CAD build for the part. Positions are in the model's coordinates, mm. Face numbers are marked on the shaded views. A direction names the side the tool comes from. Coordinates: 2 decimals unless noted, no trailing zeros. Order: outer loops, then holes, each group sorted by start corner. A loop starts at its lowest first (then second) coordinate and runs counter-clockwise, first axis right, second up. Notation, with made-up numbers: M 73,88 L 99,88 A16 cw 99,111 Z; hole C 81,35 d6. An arc over 180 degrees is marked long. Write item = value, one per line. Start each with the question number.
```python
from build123d import *

# Parameters (mm, degrees)
HUB_SKETCH_20_R            = 10
HUB_CYLINDER_20_DEPTH      = 20
FIRST_START                = -20
FIRST_ARM_DEPTH            = 20
SECOND_START               = -20
SECOND_ARM_DEPTH           = 20
TAB_A_DEPTH                = 2.5
TAB_B_DEPTH                = 2.5
TAB_B_HOLE_SKETCH_10_R     = 5
TAB_B_HOLE_10_DEPTH        = 2.5
TAB_A_HOLE_SKETCH_10_R     = 5
TAB_A_HOLE_10_DEPTH        = 2.5
HUB_CROSS_BORE_SKETCH_10_R = 5
HUB_CROSS_BORE_10_DEPTH    = 20


with BuildPart() as part:
    # Hub Sketch Ø20 → Hub Cylinder Ø20 (new body)
    with BuildSketch(Plane.XY):
        Circle(HUB_SKETCH_20_R)
    extrude(amount=HUB_CYLINDER_20_DEPTH)

    # First Arm Sketch → First Arm (add)
    with BuildSketch(Plane.XY.offset(20).offset(FIRST_START)):
        with BuildLine():
            Line((0, 10), (25, 10))
            Line((25, 10), (25, 7.5))
            Line((25, 7.5), (6.614378278, 7.5))
            ThreePointArc((6.614378278, 7.5), (3.535533906, 9.354143467), (0, 10))
        make_face()
        with BuildLine():
            Line((0, -10), (-25, -10))
            Line((-25, -10), (-25, -7.5))
            Line((-25, -7.5), (-6.614378278, -7.5))
            ThreePointArc((-6.614378278, -7.5), (-3.535533906, -9.354143467), (0, -10))
        make_face()
    extrude(amount=FIRST_ARM_DEPTH)

    # Second Arm Sketch → Second Arm (add)
    with BuildSketch(Plane.XY.offset(20).offset(SECOND_START)):
        with BuildLine():
            ThreePointArc((-9.860132972, -1.666666667), (-10.971386379, -5.727486122), (-14.790199458, -7.5))
            Line((-14.790199458, -7.5), (-6.614378278, -7.5))
            ThreePointArc((-6.614378278, -7.5), (-8.738382269, -4.86216776), (-9.860132972, -1.666666667))
        make_face()
        with BuildLine():
            ThreePointArc((9.860132972, 1.666666667), (10.971386379, 5.727486122), (14.790199458, 7.5))
            Line((14.790199458, 7.5), (6.614378278, 7.5))
            ThreePointArc((6.614378278, 7.5), (8.738382269, 4.86216776), (9.860132972, 1.666666667))
        make_face()
    extrude(amount=SECOND_ARM_DEPTH)

    # Tab A Sketch → Tab A (add)
    with BuildSketch(Plane.XZ.offset(10)):
        with BuildLine():
            Line((-25, 20), (-25, 0))
            ThreePointArc((-25, 0), (-35, 10), (-25, 20))
        make_face()
    extrude(amount=-TAB_A_DEPTH)

    # Tab B Sketch → Tab B (add)
    with BuildSketch(Plane(origin=(0, 10, 0), x_dir=(1, 0, 0), z_dir=(0, 1, 0))):
        with BuildLine():
            Line((25, 0), (25, -20))
            ThreePointArc((25, -20), (35, -10), (25, 0))
        make_face()
    extrude(amount=-TAB_B_DEPTH)

    # Tab B Hole Sketch Ø10 → Tab B Hole Ø10 (cut)
    with BuildSketch(Plane(origin=(0, 10, 0), x_dir=(1, 0, 0), z_dir=(0, 1, 0))):
        with Locations(Location((25, -10, 0), (0, 0, 270))):
            Circle(TAB_B_HOLE_SKETCH_10_R)
    extrude(amount=-TAB_B_HOLE_10_DEPTH, mode=Mode.SUBTRACT)

    # Tab A Hole Sketch Ø10 → Tab A Hole Ø10 (cut)
    with BuildSketch(Plane.XZ.offset(10)):
        with Locations(Location((-25, 10, 0), (0, 0, 270))):
            Circle(TAB_A_HOLE_SKETCH_10_R)
    extrude(amount=-TAB_A_HOLE_10_DEPTH, mode=Mode.SUBTRACT)

    # Hub Cross Bore Sketch Ø10 → Hub Cross Bore Ø10 (cut)
    with BuildSketch(Plane.XY.offset(20)):
        Circle(HUB_CROSS_BORE_SKETCH_10_R)
    extrude(amount=-HUB_CROSS_BORE_10_DEPTH, mode=Mode.SUBTRACT)


solid = part.part
```
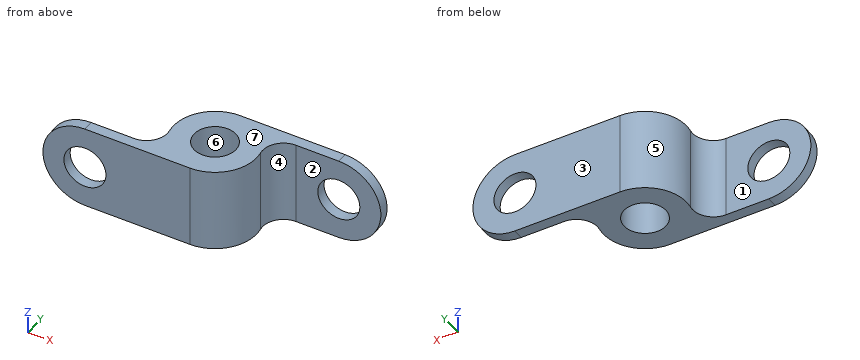
1. Flat gauge pins, fed straight in: pin 1 (6 mm diameter, centred on y = 1, z = 13.5, fed in from -X); pin 2 (1.5 mm diameter, centred on y = 3, z = 15.5, fed in from -X); pin 3 (12 mm diameter, centred on x = -7.5, z = 8.5, fed in from +Y). Where does each tip first touch, or does it go through?
2. Slice it at B-B (y = 0). Write the cut outline in (x, z), plus the area to 3 significant figures.
3. 3-axis set-ups, long thin cutter, end or side, ignore diameter. For the marked faces 1, 2 and 3: which of +Z, -Z, +X, -X, +Y, -Y reach the whole face in a straight line?
4. Mould opens along X. For the marked faces 4, 5, 6 and 7 say: released by +X, released by -X, zero draft, split by the parting line, or undercut.
5. Probe L1, parallel to X at y = 2.5, z = 11; L2, parallel to Y at x = -30, z = 12.75; L3, parallel to X at y = 0.25, z = 1.25. List the from-to ranges inside material, lowest first.
6. Slice it at A-A (z = 8.5). Write the cut outline in (x, y), plus the area to 3 significant figures.
7. Slice it at C-C (z = 1). Write the cut outline in (x, y).
8. Slice it at D-D (x = -15.5). Write the cut outline in (y, z).
Calculated:
q1.pin_1 = -10
q1.pin_2 = -9.74
q1.pin_3 = 9.89
q2.outline = M -10,0 L -5,0 L -5,20 L -10,20 Z; M 5,0 L 10,0 L 10,20 L 5,20 Z
q2.area = 200 mm²
q3.face_1 = +Z, -Z, -X, +Y
q3.face_2 = +Z, -Z, +X, -Y
q3.face_3 = +Z, -Z, +X, -X, +Y
q4.face_4 = released by +X
q4.face_5 = released by -X
q4.face_6 = undercut
q4.face_7 = zero draft
q5.L1 = -9.68 to -4.33, 4.33 to 9.79
q5.L2 = -10 to -7.5
q5.L3 = -10 to -4.99, 4.99 to 10
q6.outline = M -34.89,-10 L -29.77,-10 L -29.77,-7.5 L -34.89,-7.5 Z; M -20.23,-10 L 0,-10 A10 ccw 9.86,1.67 A5 cw 14.79,7.5 L 20.23,7.5 L 20.23,10 L 0,10 A10 ccw -9.86,-1.67 A5 cw -14.79,-7.5 L -20.23,-7.5 Z; M 29.77,7.5 L 34.89,7.5 L 34.89,10 L 29.77,10 Z; hole C 0,0 d10
q6.area = 363 mm²
q7.outline = M -29.36,-10 L 0,-10 A10 ccw 9.86,1.67 A5 cw 14.79,7.5 L 29.36,7.5 L 29.36,10 L 0,10 A10 ccw -9.86,-1.67 A5 cw -14.79,-7.5 L -29.36,-7.5 Z; hole C 0,0 d10
q8.outline = M -10,0 L -7.5,0 L -7.5,20 L -10,20 Z
